from build123d import *

# Parameters (mm, degrees)
SKETCH_1_R          = 17.5
EXTRUDE_1_DEPTH     = 5
SKETCH_2_R          = 7.5
EXTRUDE_2_DEPTH     = 90.91
SKETCH_3_R          = 1.65
SKETCH_3_R_2        = 3.5
CUT_EXTRUDE_1_DEPTH = 1000
SKETCH_4_R          = 10
SKETCH_4_R_2        = 4
EXTRUDE_3_DEPTH     = 15.66
SKETCH_5_R          = 1.65
CUT_EXTRUDE_2_DEPTH = 8


with BuildPart() as part:
    # 草图1 → 凸台-拉伸1 (new body)
    with BuildSketch(Plane.XY):
        Circle(SKETCH_1_R)
    extrude(amount=EXTRUDE_1_DEPTH)

    # 草图2 → 凸台-拉伸2 (add)
    with BuildSketch(Plane.XY.offset(5)):
        Circle(SKETCH_2_R)
    extrude(amount=EXTRUDE_2_DEPTH)

    # 草图3 → 切除-拉伸1 (cut)
    with BuildSketch(Plane(origin=(0, 0, 0), x_dir=(-1, 0, 0), z_dir=(0, 0, -1))):
        with Locations((0, 13.5)):
            Circle(SKETCH_3_R)
        with Locations((11.691342951, 6.75)):
            Circle(SKETCH_3_R)
        with Locations((11.691342951, -6.75)):
            Circle(SKETCH_3_R)
        with Locations((0, -13.5)):
            Circle(SKETCH_3_R)
        with Locations((-11.691342951, -6.75)):
            Circle(SKETCH_3_R)
        with Locations((-11.691342951, 6.75)):
            Circle(SKETCH_3_R)
        Circle(SKETCH_3_R_2)
    extrude(amount=-CUT_EXTRUDE_1_DEPTH, mode=Mode.SUBTRACT)

    # 草图4 → 凸台-拉伸3 (add)
    with BuildSketch(Plane.XY.offset(95.91)):
        Circle(SKETCH_4_R)
        Circle(SKETCH_4_R_2, mode=Mode.SUBTRACT)
    extrude(amount=-EXTRUDE_3_DEPTH)

    # 草图5 → 切除-拉伸2 (cut)
    with BuildSketch(Plane.XY.offset(95.91)):
        with Locations((-4.242640687, 4.242640687)):
            Circle(SKETCH_5_R)
        with Locations((-4.242640687, -4.242640687)):
            Circle(SKETCH_5_R)
        with Locations((4.242640687, -4.242640687)):
            Circle(SKETCH_5_R)
        with Locations((4.242640687, 4.242640687)):
            Circle(SKETCH_5_R)
    extrude(amount=-CUT_EXTRUDE_2_DEPTH, mode=Mode.SUBTRACT)


solid = part.part
Work out the finished part from the listing and answer in its coordinate system (mm). A direction names the side the tool comes from. Coordinates: 2 decimals unless noted, no trailing zeros. Write each loop counter-clockwise with the first axis right and the second up, starting at its lowest first coordinate (ties: lowest second). Pieces come first, ordered by that corner, then holes. Notation, with made-up numbers: (-26.5, 19) - (-2.5, 19) arc R20 ccw to (-2.5, 46) - close; hole circle Ø10 at (13.5, 78). An arc over 180 degrees is marked (long way). One line per question, with ' | ' between items.
1) Find section A-A, the plane y = 0. Determine the outline of the cut face in (x, z), and give its area (3 significant figures).
Checks:
outline: (-17.5, 0) - (-3.5, 0) - (-3.5, 95.91) - (-10, 95.91) - (-10, 80.25) - (-7.5, 80.25) - (-7.5, 5) - (-17.5, 5) - close; (3.5, 0) - (17.5, 0) - (17.5, 5) - (7.5, 5) - (7.5, 80.25) - (10, 80.25) - (10, 95.91) - (3.5, 95.91) - close | area: 946 mm2
2) Find section B-B, the plane x = 0. Determine the outline of the cut face in (y, z), and give its area (3 significant figures).
Checks:
outline: (-17.5, 0) - (-15.15, 0) - (-15.15, 5) - (-17.5, 5) - close; (-11.85, 0) - (-3.5, 0) - (-3.5, 95.91) - (-10, 95.91) - (-10, 80.25) - (-7.5, 80.25) - (-7.5, 5) - (-11.85, 5) - close; (3.5, 0) - (11.85, 0) - (11.85, 5) - (7.5, 5) - (7.5, 80.25) - (10, 80.25) - (10, 95.91) - (3.5, 95.91) - close; (15.15, 0) - (17.5, 0) - (17.5, 5) - (15.15, 5) - close | area: 913 mm2
3) Find section C-C, the plane z = 27. Determine the outline of the cut face in (x, y), and give its area (3 significant figures).
Checks:
outline: circle Ø15 at (0, 0); hole circle Ø7 at (0, 0) | area: 138 mm2
4) The mould has two halves that part along Y. Classify faces 4 (the face through (-2.17, -9.76, 88.19)), 5 (the face through (0, -8, 5)), 6 (the face through (2.93, 3.24, 91.97)): +Y half, -Y half, draft (parallel to the pull), parting line (faces both ways), or undercut.
Checks:
face 4: parting line | face 5: draft | face 6: undercut
5) For faces 1 (the face through (-3.233, -1.341, 47.284)), 2 (the face through (-7.493, 0.33, 42.098)), 3 (the face through (4, 4, 87.91)), determine the directions among +Z, -Z, +X, -X, +Y, -Y from which every point of the face is accessible in a straight line to the end or side of a thin tool.
Checks:
face 1: +Z, -Z | face 2: none | face 3: +Z
6) Find section D-D, the plane x = 11. Determine the outline of the cut face in (y, z).
Checks:
outline: (-13.61, 0) - (-8.25, 0) - (-8.25, 5) - (-13.61, 5) - close; (-5.25, 0) - (5.25, 0) - (5.25, 5) - (-5.25, 5) - close; (8.25, 0) - (13.61, 0) - (13.61, 5) - (8.25, 5) - close
7) Flat-ended cylindrical pins translate along their axes: P1, Ø5.5, axis at x = -4.24, y = 4.24, coming from the +Z side; P2, Ø6, axis at y = -9.5, z = 17.5, coming from the +X side; P3, Ø8, axis at x = 2, z = 86.5, coming from the +Y side; P4, Ø4, axis at y = -4, z = 58, coming from the -X side. Find the tip coordinate at first contact, or state that the pin passes through.
Checks:
P1: z = 95.91 | P2: x = 3.74 | P3: y = 10 | P4: x = -7.23
8) Consider probe 1 along Y at (x, z) = (0, 3.8); probe 2 along Y at (x, z) = (0, 54); probe 3 along Z at (x, y) = (1.5, 7.5). Determine where each line is inside the solid, lowest interval first. Write a range as [from, to].
Checks:
probe 1: [-17.5, -15.15], [-11.85, -3.5], [3.5, 11.85], [15.15, 17.5] | probe 2: [-7.5, -3.5], [3.5, 7.5] | probe 3: [0, 5], [80.25, 95.91]
